Geometry: see drawing. Coordinates: mm, zero at the bounding-box minimum. A direction names the side the tool comes from. Coordinates: 2 decimals unless noted, no trailing zeros. Loops run counter-clockwise (first coordinate to the right, second up) from the corner with the lowest first, then second, coordinate; pieces in that order, holes last.
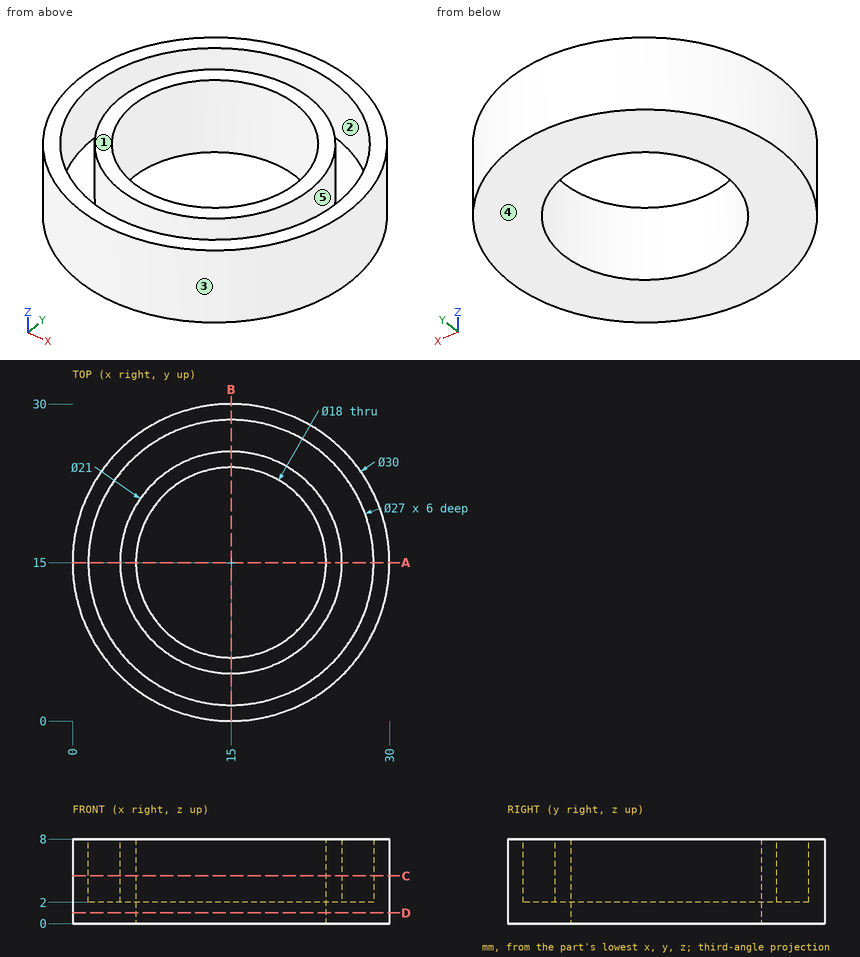
Item 1: Section query A-A (y = 15). Output: boundary loops of the cut face in (x, z), then the cut area to 3 significant figures.
Result:
outline: (0, 0) - (6, 0) - (6, 8) - (4.5, 8) - (4.5, 2) - (1.5, 2) - (1.5, 8) - (0, 8) - close; (24, 0) - (30, 0) - (30, 8) - (28.5, 8) - (28.5, 2) - (25.5, 2) - (25.5, 8) - (24, 8) - close
area: 60.0 mm2
Item 2: Reachability of the marked faces 4 and 5 from +Z, -Z, +X, -X, +Y, -Y: full face, straight path, thin tool, end or side. Return the list, or none.
Result:
face 4: -Z, +X, -X, +Y, -Y
face 5: +Z
Item 3: Section query C-C (z = 4.5). Output: boundary loops of the cut face in (x, y).
Result:
outline: circle Ø30 at (15, 15); circle Ø21 at (15, 15); hole circle Ø27 at (15, 15); hole circle Ø18 at (15, 15)
Item 4: Contact query for flat-ended pins moving along their axis: P1, Ø1.5, axis at x = 9.5, y = 3.5, coming from the -Z side; P2, Ø3, axis at x = 11, z = 5.5, coming from the -Y side; P3, Ø4, axis at x = 19, z = 3, coming from the -Y side. Output: stop coordinate, or through.
Result:
P1: stops at z = 0
P2: stops at y = 0.21
P3: stops at y = 0.13
Item 5: Mould query, pull axis X, two halves, no side actions, for the marked faces 1, 2 and 3. Classes: +X half, -X half, draft (parallel to the pull), parting line (faces both ways), or undercut.
Result:
face 1: draft
face 2: undercut
face 3: parting line
Item 6: Section query D-D (z = 1). Output: boundary loops of the cut face in (x, y), then the cut area to 3 significant figures.
Result:
outline: circle Ø30 at (15, 15); hole circle Ø18 at (15, 15)
area: 452 mm2
Item 7: Line query: L1, parallel to Y at x = 15, z = 3; L2, parallel to Y at x = 17.5, z = 6; L3, parallel to X at y = 21, z = 2.25. Output: solid intervals per line, ascending.
Result:
L1: y = 0 to 1.5, 4.5 to 6, 24 to 25.5, 28.5 to 30
L2: y = 0.21 to 1.73, 4.8 to 6.35, 23.65 to 25.2, 28.27 to 29.79
L3: x = 1.25 to 2.91, 6.38 to 8.29, 21.71 to 23.62, 27.09 to 28.75
